Can you work these out from the model? Positions are in its coordinate system, mm. Face numbers are marked on the shaded views. A direction names the side the tool comes from. Give positions to 0.01 mm unless a question says otherwise; leave off trailing zeros. Loops run counter-clockwise (first coordinate to the right, second up) from the corner with the lowest first, then second, coordinate; pieces in that order, holes last. Notation, with made-up numbers: (1, 0) - (58, 0) arc R22 cw to (58, 36) - close; hole circle Ø8 at (85, 59). An arc over 180 degrees is marked (long way). Answer as a JSON object with one key per item and string values.
```python
from build123d import *

# Parameters (mm, degrees)
L_STRIP_BODY_DEPTH         = 10.5
EYE_LUG_A_SKETCH_R         = 20
EYE_LUG_A_40_DEPTH         = 7
EYE_HOLE_A_18_DEPTH        = 7
EYE_LUG_B_SKETCH_R         = 20
EYE_LUG_B_SKETCH_R_2       = 9
EYE_LUG_B_40_DEPTH         = 7
EYE_HOLE_B_18_DEPTH        = 7
OUTER_BEND_FILLET_R14_R    = 14
INNER_BEND_FILLET_R7_R     = 7
EYE_LUG_BLEND_FILLETS_R5_R = 5


with BuildPart() as part:
    # L Strip Profile Sketch → L Strip Body (new, symmetric)
    with BuildSketch(Plane.XY):
        Polygon((85, 0), (0, 0), (0, -55), (7, -55), (7, -7), (85, -7), align=None)
    extrude(amount=L_STRIP_BODY_DEPTH, both=True)

    # Eye Lug A Sketch → Eye Lug A _40 (add)
    with BuildSketch(Plane(origin=(0, 0, 0), x_dir=(1, 0, 0), z_dir=(0, 1, 0))):
        with Locations((85, 0)):
            Circle(EYE_LUG_A_SKETCH_R)
    extrude(amount=-EYE_LUG_A_40_DEPTH)

    # Sketch2_3 → Eye Hole A _18 (cut)
    with BuildSketch(Plane(origin=(0, 0, 0), x_dir=(1, 0, 0), z_dir=(0, 1, 0))):
        with BuildLine():
            Line((85, 9), (85, -9))
            ThreePointArc((85, -9), (91.363961031, -6.363961031), (94, 0))
            ThreePointArc((94, 0), (91.363961031, 6.363961031), (85, 9))
        make_face()
        with BuildLine():
            ThreePointArc((85, 9), (76, 0), (85, -9))
            Line((85, -9), (85, 9))
        make_face()
        with BuildLine():
            Line((85, 9), (85, -9))
            ThreePointArc((85, -9), (91.363961031, -6.363961031), (94, 0))
            ThreePointArc((94, 0), (91.363961031, 6.363961031), (85, 9))
        make_face()
        with BuildLine():
            ThreePointArc((85, 9), (76, 0), (85, -9))
            Line((85, -9), (85, 9))
        make_face()
    extrude(amount=-EYE_HOLE_A_18_DEPTH, mode=Mode.SUBTRACT)

    # Eye Lug B Sketch → Eye Lug B _40 (add)
    with BuildSketch(Plane.ZY):
        with Locations((0, -55)):
            Circle(EYE_LUG_B_SKETCH_R)
        with Locations((0, -55)):
            Circle(EYE_LUG_B_SKETCH_R_2, mode=Mode.SUBTRACT)
    extrude(amount=-EYE_LUG_B_40_DEPTH)

    # Sketch4_2 → Eye Hole B _18 (cut)
    with BuildSketch(Plane.ZY):
        with BuildLine():
            Line((-9, -55), (9, -55))
            ThreePointArc((9, -55), (0, -46), (-9, -55))
        make_face()
        with BuildLine():
            ThreePointArc((-9, -55), (0, -64), (9, -55))
            Line((9, -55), (-9, -55))
        make_face()
    extrude(amount=-EYE_HOLE_B_18_DEPTH, mode=Mode.SUBTRACT)

    # Outer Bend Fillet R14
    outer_bend_fillet_r14_edges = [part.edges().sort_by_distance(p)[0] for p in [
        (0, 0, 0),
    ]]
    fillet(outer_bend_fillet_r14_edges, radius=OUTER_BEND_FILLET_R14_R)

    # Inner Bend Fillet R7
    inner_bend_fillet_r7_edges = [part.edges().sort_by_distance(p)[0] for p in [
        (7, -7, 0),
    ]]
    fillet(inner_bend_fillet_r7_edges, radius=INNER_BEND_FILLET_R7_R)

    # Eye Lug Blend Fillets R5
    eye_lug_blend_fillets_r5_edges = [part.edges().sort_by_distance(p)[0] for p in [
        (67.977955469, -3.5, 10.5),
        (67.977955469, -3.5, -10.5),
        (3.5, -37.977955469, -10.5),
        (3.5, -37.977955469, 10.5),
    ]]
    fillet(eye_lug_blend_fillets_r5_edges, radius=EYE_LUG_BLEND_FILLETS_R5_R)


solid = part.part
```
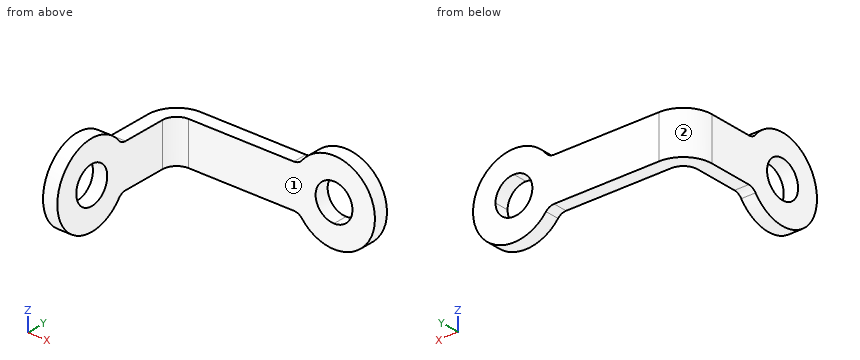
1) Imagine slicing it at A-A on y = -55. Write out the boundary of the cut face in (x, z), and give its area (3 significant figures).
Check sheet entries:
{"outline": "(0, -20) - (7, -20) - (7, -9) - (0, -9) - close; (0, 9) - (7, 9) - (7, 20) - (0, 20) - close", "area": "154 mm2"}
2) Imagine slicing it at B-B on x = 82. Write out the boundary of the cut face in (y, z).
Check sheet entries:
{"outline": "(-7, -19.77) - (0, -19.77) - (0, -8.49) - (-7, -8.49) - close; (-7, 8.49) - (0, 8.49) - (0, 19.77) - (-7, 19.77) - close"}
3) I need wall thicknesses on L1, parallel to Y at x = 22.5, z = 4; L2, parallel to X at y = -47, z = 11; L3, parallel to Y at x = 3.5, z = 0. Which ranges of each line are inside material? Lowest first, please.
Check sheet entries:
{"L1": "-7 to 0", "L2": "0 to 7", "L3": "-75 to -64, -46 to -4.74"}
4) Imagine slicing it at D-D on y = -27.5. Write out the boundary of the cut face in (x, z).
Check sheet entries:
{"outline": "(0, -10.5) - (7, -10.5) - (7, 10.5) - (0, 10.5) - close"}
5) Imagine slicing it at C-C on z = 4. Write out the boundary of the cut face in (x, y).
Check sheet entries:
{"outline": "(0, -74.6) - (7, -74.6) - (7, -63.06) - (0, -63.06) - close; (0, -46.94) - (7, -46.94) - (7, -14) arc R7 cw to (14, -7) - (76.94, -7) - (76.94, 0) - (14, 0) arc R14 ccw to (0, -14) - close; (93.06, -7) - (104.6, -7) - (104.6, 0) - (93.06, 0) - close"}
6) I'm going to push flat-ended pins straight in: P1, Ø3, axis at x = 78.5, z = -4.5, coming from the -Y side; P2, Ø8, axis at y = -16, z = -4, coming from the +X side; P3, Ø12, axis at y = -45.5, z = 3.5, coming from the +X side. Where does each tip first touch, or does it pass through?
Check sheet entries:
{"P1": "y = -7", "P2": "x = 7.29", "P3": "x = 7"}
7) Which directions (+Z, -Z, +X, -X, +Y, -Y) give clear straight access to the entire face, cutting with the end or side of a thin tool? Please do the marked faces 1 and 2.
Check sheet entries:
{"face 1": "+Z, -Z, +X, -Y", "face 2": "+Z, -Z, -X, +Y"}
